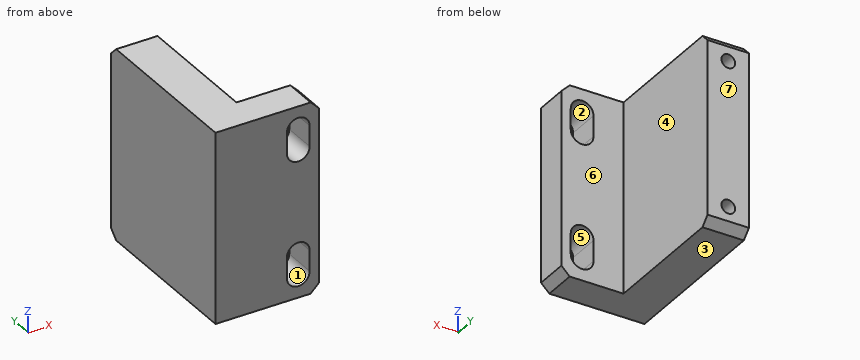
```python
from build123d import *

# Parameters (mm, degrees)
BOSS_EXTRUDE1_DEPTH   = 23
CUT_EXTRUDE1_DEPTH    = 54.244718048
M4_TAPPED_HOLE1_D     = 3.3
M4_TAPPED_HOLE1_DEPTH = 10.1
M4_TAPPED_HOLE1_TIP   = 0.991420021
CHAMFER4_SIZE         = 2


with BuildPart() as part:
    # Sketch1 → Boss-Extrude1 (new, symmetric)
    with BuildSketch(Plane.XY):
        Polygon((0, 41), (10, 41), (10, 8), (25, 8), (25, 0), (0, 0), align=None)
    extrude(amount=BOSS_EXTRUDE1_DEPTH, both=True)

    # Sketch2 → Cut-Extrude1 (cut, through all)
    with BuildSketch(Plane(origin=(0, 0, 0), x_dir=(1, 0, 0), z_dir=(0, 1, 0))):
        with BuildLine():
            Line((22.75, 17.5), (22.75, 12.5))
            ThreePointArc((22.75, 12.5), (20, 9.75), (17.25, 12.5))
            Line((17.25, 12.5), (17.25, 17.5))
            ThreePointArc((17.25, 17.5), (20, 20.25), (22.75, 17.5))
        make_face()
        with BuildLine():
            Line((22.75, -12.5), (22.75, -17.5))
            ThreePointArc((22.75, -17.5), (20, -20.25), (17.25, -17.5))
            Line((17.25, -17.5), (17.25, -12.5))
            ThreePointArc((17.25, -12.5), (20, -9.75), (22.75, -12.5))
        make_face()
    extrude(amount=CUT_EXTRUDE1_DEPTH, mode=Mode.SUBTRACT)

    # M4 Tapped Hole1
    with Locations(Plane(origin=(0, 41, 0), x_dir=(1, 0, 0), z_dir=(0, 1, 0))):
        with Locations((5, 17.5), (5, -17.5)):
            Hole(M4_TAPPED_HOLE1_D / 2, depth=M4_TAPPED_HOLE1_DEPTH)
            with Locations((0, 0, -(M4_TAPPED_HOLE1_DEPTH + M4_TAPPED_HOLE1_TIP / 2))):  # 118° drill point
                Cone(0, M4_TAPPED_HOLE1_D / 2, M4_TAPPED_HOLE1_TIP, mode=Mode.SUBTRACT)

    # Chamfer4
    chamfer4_edges = [part.edges().sort_by_distance(p)[0] for p in [
        (25, 4, 23),
        (5, 41, 23),
        (5, 41, -23),
        (25, 4, -23),
    ]]
    chamfer(chamfer4_edges, length=CHAMFER4_SIZE)


solid = part.part
```
Geometry check sheet. Reference: the model listing, model coordinates, mm. Face numbers are marked on the shaded views. A direction names the side the tool comes from. Coordinates: 2 decimals unless noted, no trailing zeros. Loops run counter-clockwise (first coordinate to the right, second up) from the corner with the lowest first, then second, coordinate; pieces in that order, holes last.
Item 1: Sectioned sample at C-C, the plane z = -11. Record the boundary of the cut face in (x, y), then the cut area to 3 significant figures.
Item 2: Release check for a two-part mould opening along X. For the marked faces 1, 2, 3 and 4 record: released by +X, released by -X, zero draft, split by the parting line, or undercut.
Item 3: Sectioned sample at D-D, the plane z = -4.5. Record the boundary of the cut face in (x, y).
Item 4: Access from +Z, -Z, +X, -X, +Y, -Y to the whole of each face (thin tool, end or side, straight path). Record for the marked faces 5, 6 and 7.
Item 5: Sectioned sample at A-A, the plane x = 20. Record the boundary of the cut face in (y, z).
Item 6: Thickness scan on line 1 (Z direction, x = 5, y = 35.25); line 2 (X direction, y = 36, z = -17.5); line 3 (X direction, y = 25.5, z = 14). Record the ranges inside material, lowest first.
Item 7: Go/stop test with flat-tipped pins: pin 1 Ø12 at (x, y) = (17, 33.5) entering from +Z; pin 2 Ø2.5 at (x, z) = (5, -17.5) entering from -Y; pin 3 Ø12 at (x, z) = (20.5, -9.5) entering from +Y. Record where each tip stops, or that it passes through.
Item 8: Sectioned sample at B-B, the plane y = 7. Record the boundary of the cut face in (x, z).
Check result:
1. outline: (0, 0) - (17.7, 0) - (17.7, 8) - (10, 8) - (10, 41) - (0, 41) - close; (22.3, 0) - (25, 0) - (25, 8) - (22.3, 8) - close
1. area: 493 mm2
2. face 1: undercut
2. face 2: undercut
2. face 3: zero draft
2. face 4: released by +X
3. outline: (0, 0) - (25, 0) - (25, 8) - (10, 8) - (10, 41) - (0, 41) - close
4. face 5: +Y, -Y
4. face 6: +Z, -Z, +X, +Y
4. face 7: +Z, -Z, +X, -X, +Y
5. outline: (0, -23) - (8, -23) - (8, -20.25) - (0, -20.25) - close; (0, -9.75) - (8, -9.75) - (8, 9.75) - (0, 9.75) - close; (0, 20.25) - (8, 20.25) - (8, 23) - (0, 23) - close
6. line 1: z = -23 to -19.15, -15.85 to 15.85, 19.15 to 23
6. line 2: x = 0 to 3.35, 6.65 to 10
6. line 3: x = 0 to 10
7. pin 1: passes through
7. pin 2: stops at y = 0
7. pin 3: stops at y = 8
8. outline: (0, -23) - (23, -23) - (25, -21) - (25, 21) - (23, 23) - (0, 23) - close; hole (17.25, -17.5) arc R2.75 ccw to (22.75, -17.5) - (22.75, -12.5) arc R2.75 ccw to (17.25, -12.5) - close; hole (17.25, 12.5) arc R2.75 ccw to (22.75, 12.5) - (22.75, 17.5) arc R2.75 ccw to (17.25, 17.5) - close
